Part model, mm, in its own coordinate system. Coordinates: 2 decimals unless noted, no trailing zeros. Write each loop counter-clockwise with the first axis right and the second up, starting at its lowest first coordinate (ties: lowest second). Pieces come first, ordered by that corner, then holes. Notation, with made-up numbers: (78.25, 25.5) - (99.25, 25.5) arc R9 cw to (99.25, 37.5) - close; hole circle Ø4 at (-0.5, 46.5). An arc over 180 degrees is marked (long way). Write each question's results on one line, items separated by ' | '.
from build123d import *

# Parameters (mm, degrees)
SKETCH_1_W          = 12
SKETCH_1_H          = 60
EXTRUDE_1_DEPTH     = 6
SKETCH_2_W          = 10
SKETCH_2_H          = 60
CUT_EXTRUDE_1_DEPTH = 0.75


with BuildPart() as part:
    # 草图1 → 凸台-拉伸1 (new body)
    with BuildSketch(Plane(origin=(0, 0, 0), x_dir=(1, 0, 0), z_dir=(0, 1, 0))):
        Rectangle(SKETCH_1_W, SKETCH_1_H)
    extrude(amount=EXTRUDE_1_DEPTH)

    # 草图2 → 切除-拉伸1 (cut)
    with BuildSketch(Plane(origin=(0, 6, 0), x_dir=(1, 0, 0), z_dir=(0, 1, 0))):
        Rectangle(SKETCH_2_W, SKETCH_2_H)
    extrude(amount=-CUT_EXTRUDE_1_DEPTH, mode=Mode.SUBTRACT)


solid = part.part
(1) Saw through at A-A on z = -6. Write the cut outline in (x, y).
Return value:
outline: (-6, 0) - (6, 0) - (6, 6) - (5, 6) - (5, 5.25) - (-5, 5.25) - (-5, 6) - (-6, 6) - close
(2) Wall check: line 1 (X direction, y = 5.3, z = -8); line 2 (Y direction, x = 2, z = -5). Give the ranges that are in metal, low to high. Write a range as from..to.
Return value:
line 1: x = -6..-5, 5..6 | line 2: y = 0..5.25
(3) Flat gauge pin, fed straight in: P1, Ø5, axis at x = 0, z = 13, coming from the +Y side. Where does the tip first touch, or does it go through?
Return value:
P1: stops at y = 5.25
(4) Two-plate mould, pull along X, no slides. Class faces 1 (the flat face through (-6, 3, 0)), 2 (the flat face through (-5.5, 6, -0.4)), 3 (the flat face through (0, 5.25, 0)): released by +X, released by -X, zero draft, split by the parting line, or undercut.
Return value:
face 1: released by -X | face 2: zero draft | face 3: undercut
(5) Saw through at B-B on x = -3.5. Write the cut outline in (y, z).
Return value:
outline: (0, -30) - (5.25, -30) - (5.25, 30) - (0, 30) - close
